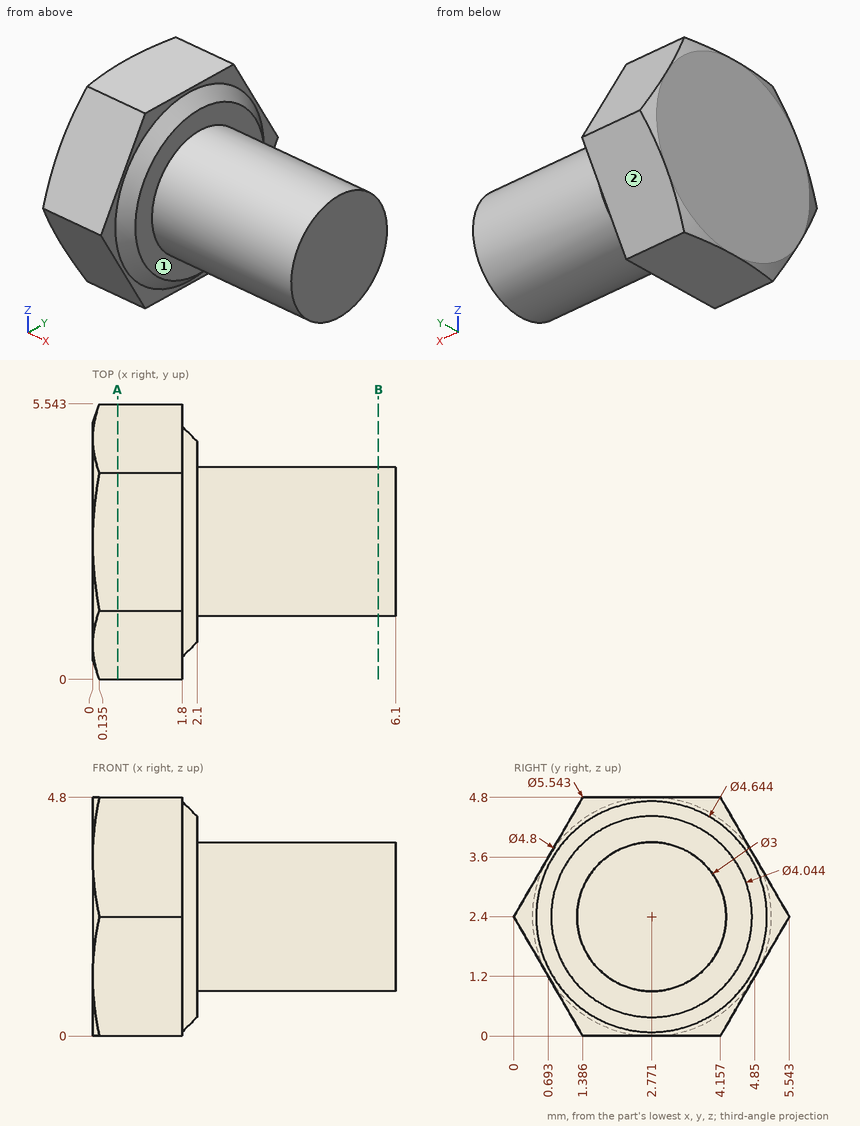
Part print with two shaded views. Sizes in mm from the minimum x, y, z corner. A direction names the side the tool comes from. Coordinates: 2 decimals unless noted, no trailing zeros. Write each loop counter-clockwise with the first axis right and the second up, starting at its lowest first coordinate (ties: lowest second). Pieces come first, ordered by that corner, then holes. Notation, with made-up numbers: (-12, 13.5) -> (32, 13.5) arc R24 ccw to (32, 28.5) -> close; hole circle Ø11 at (66, -15.5). An arc over 180 degrees is marked (long way). Return JSON: item names as keys, results as strings. Group by question number.
Q1. Drill centre lines: line 1 (X direction, y = 3.7, z = 3.7); line 2 (Y direction, x = 2.25, z = 3.45) (1 decimal); line 3 (Z direction, x = 4.5, y = 2.7). Where is each one in solid material? Low to high.
Q2. Cut at B-B, the plane x = 5.75. Give the cut face in (y, z).
Q3. Which spindle directions (+Z, -Z, +X, -X, +Y, -Y) get a long thin tool onto all of the face, cutting with end or side? Do the marked faces 1 and 2. Say none if no direction does.
Q4. Cut at A-A, the plane x = 0.5. Give the cut face in (y, z) (1 decimal).
Q5. Flat gauge pins, fed straight in: pin 1 (3 mm diameter, centred on x = 4, y = 2.5, fed in from -Z); pin 2 (1 mm diameter, centred on x = 1, z = 4, fed in from -Y) (1 decimal); pin 3 (1 mm diameter, centred on x = 5, z = 3.5, fed in from -Y). Where does each tip first touch, or does it go through?
Returned:
{
 "1": {"line 1": "x = 0 to 2.1", "line 2": "y = 1.7 to 3.8", "line 3": "z = 0.9 to 3.9"},
 "2": {"outline": "circle Ø3 at (2.77, 2.4)"},
 "3": {"face 1": "+X", "face 2": "-Z, +X, -X, +Y"},
 "4": {"outline": "(0, 2.4) -> (1.4, 0) -> (4.2, 0) -> (5.5, 2.4) -> (4.2, 4.8) -> (1.4, 4.8) -> close"},
 "5": {"pin 1": "stops at z = 0.9", "pin 2": "stops at y = 0.6", "pin 3": "stops at y = 1.4"}
}
